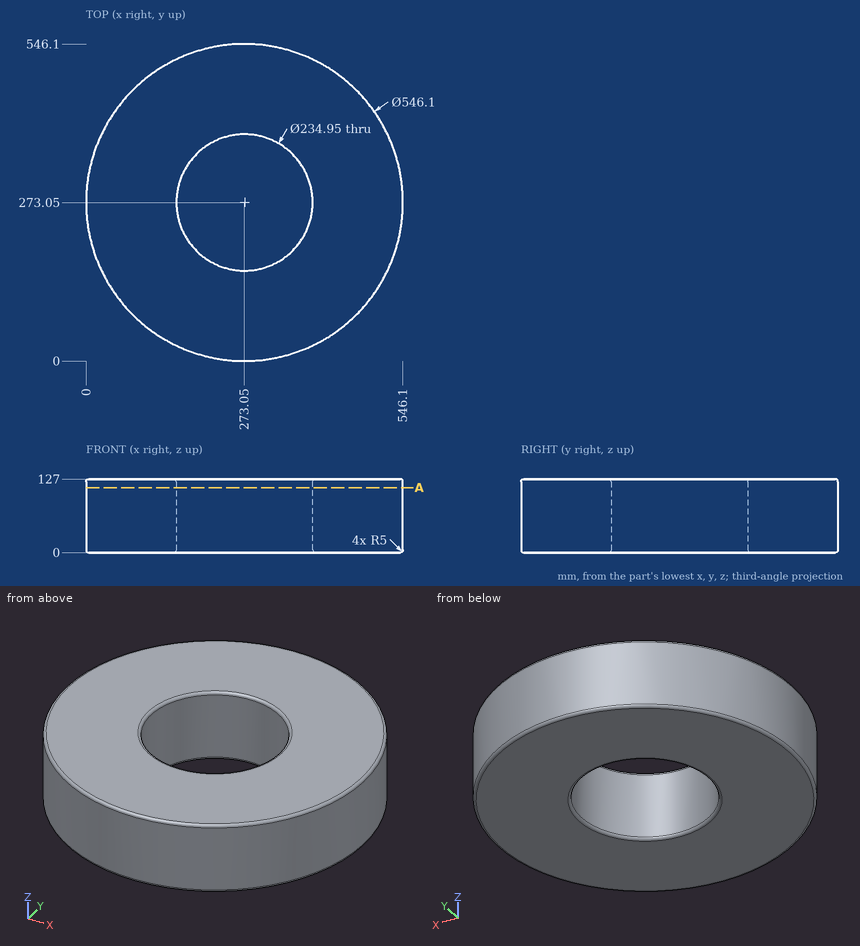
The figure shows three views and two pictorial views of one solid part (mm, origin at its lowest corner). Answer the questions. Give positions to 0.01 mm unless a question says otherwise; leave off trailing zeros. Write each loop counter-clockwise with the first axis right and the second up, starting at its lowest first coordinate (ties: lowest second). Pieces come first, ordered by that corner, then holes. Notation, with made-up numbers: M -34.75,72.25 L 4.25,72.25 A36 cw 4.25,109.25 Z; hole C 65.5,87.5 d3. An arc over 180 degrees is marked long. One line per item, written item: value. Start each with the question number.
(1) Find the intervals of material crossed by line 1 (Y direction, x = 273.05, z = 44) (3 decimals); line 2 (Y direction, x = 370, z = 64); line 3 (X direction, y = 333, z = 114), in increasing order.
(2) Find section A-A (z = 112). Determine the outline of the cut face in (x, y) (3 decimals), plus the area to 3 significant figures.
(3) Flat-ended cylindrical pins translate along their axes: pin 1 Ø3 at (x, z) = (116.5, 87) entering from -Y; pin 2 Ø10 at (x, y) = (392.5, 303.5) entering from -Z; pin 3 Ø12 at (x, z) = (136.5, 14.5) entering from -Y; pin 4 Ø5 at (x, z) = (460, 91) entering from -Y. Find the tip coordinate at first contact, or state that the pin passes through.
Results below:
1. line 1: y = 0 to 155.575, 390.525 to 546.1
1. line 2: y = 17.79 to 206.71, 339.39 to 528.31
1. line 3: x = 6.66 to 172.02, 374.08 to 539.44
2. outline: C 273.05,273.05 d546.1; hole C 273.05,273.05 d234.95
2. area: 191,000 mm^2
3. pin 1: stops at y = 48.29
3. pin 2: stops at z = 0
3. pin 3: stops at y = 33.23
3. pin 4: stops at y = 71.72
